```python
from build123d import *

# Parameters (mm, degrees)
SKETCH_1_W      = 30
SKETCH_1_H      = 30
SKETCH_1_W_2    = 26
SKETCH_1_H_2    = 26
EXTRUDE_1_DEPTH = 650


with BuildPart() as part:
    # 草图1 → 凸台-拉伸1 (new, symmetric)
    with BuildSketch(Plane.XY):
        Rectangle(SKETCH_1_W, SKETCH_1_H)
        Rectangle(SKETCH_1_W_2, SKETCH_1_H_2, mode=Mode.SUBTRACT)
    extrude(amount=EXTRUDE_1_DEPTH, both=True)


solid = part.part
```
The listing builds one solid part. Answer for the finished solid, in the listing's coordinates (mm). A direction names the side the tool comes from. Coordinates: 2 decimals unless noted, no trailing zeros. Write each loop counter-clockwise with the first axis right and the second up, starting at its lowest first coordinate (ties: lowest second). Pieces come first, ordered by that corner, then holes. Notation, with made-up numbers: M 7.25,46 L 62.25,46 A25 ccw 62.25,73 Z; hole C 30.25,36.25 d5. An arc over 180 degrees is marked long. Use a Markdown table: item, result. Add a question column.
1. Section A-A (y = 8.5) is taken. Give the vertices of the cut face in (x, z).
2. Section C-C (z = -128.5) is taken. Give the vertices of the cut face in (x, y).
3. A straight line is drawn through the part: line 1 along Y through (x, z) = (6.5, 156.5). Find the intervals that lie inside material, in ascending order. Write a range as [from, to].
4. Which of the six approach directions +Z, -Z, +X, -X, +Y, -Y give full straight-line access (tool end or side, diameter ignored) to faces 1 (the flat face through (-13, 0, 9)), 2 (the flat face through (0, 15, 9))?
5. For a pull along X with two mould halves and no side action, classify faces 3 (the flat face through (0, -15, 9)), 4 (the flat face through (-15, 0, 9)), 5 (the flat face through (13, 0, 9)) as +X half, -X half, draft (parallel to the pull), parting line (faces both ways), or undercut.
Data:
| question | item | result |
|---|---|---|
| 1 | outline | M -15,-650 L -13,-650 L -13,650 L -15,650 Z; M 13,-650 L 15,-650 L 15,650 L 13,650 Z |
| 2 | outline | M -15,-15 L 15,-15 L 15,15 L -15,15 Z; hole M -13,-13 L 13,-13 L 13,13 L -13,13 Z |
| 3 | line 1 | y = [-15, -13], [13, 15] |
| 4 | face 1 | +Z, -Z |
| 4 | face 2 | +Z, -Z, +X, -X, +Y |
| 5 | face 3 | draft |
| 5 | face 4 | -X half |
| 5 | face 5 | undercut |
